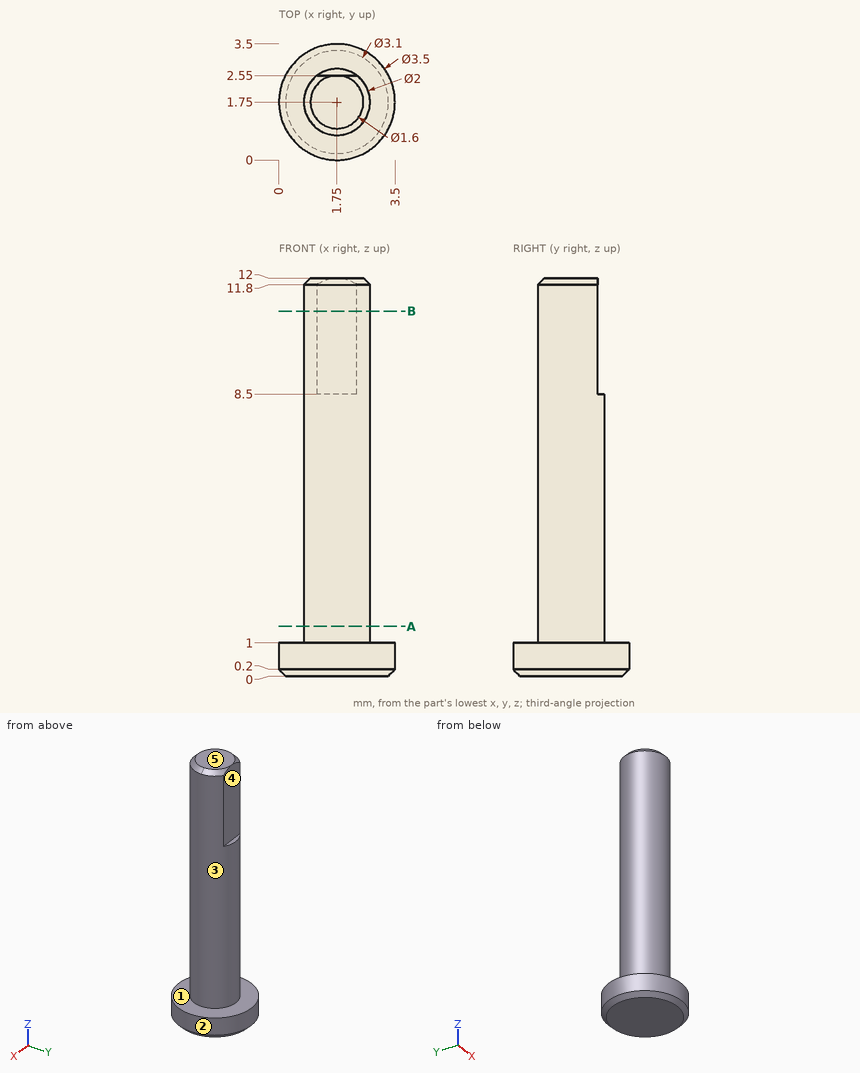
Design review of the part shown in the three views and the two pictorial views. Dimensions are in mm from the part's minimum x, y and z. A direction names the side the tool comes from. Round coordinates to 2 decimals unless told otherwise and drop trailing zeros. Loops run counter-clockwise (first coordinate to the right, second up) from the corner with the lowest first, then second, coordinate; pieces in that order, holes last. Notation, with made-up numbers: M 88,15.5 L 101,15.5 A35 ccw 101,53.5 Z; hole C -38.75,40 d10. An arc over 180 degrees is marked long. Answer as a JSON object with one key per item and string values.
Item 1: Wall thickness on L1, parallel to Y at x = 2.55, z = 8; L2, parallel to Z at x = 2.8, y = 1.35; L3, parallel to X at y = 1.65, z = 3.5: over which ranges is each line inside the solid? List them lowest first. Write a range as from..to.
Answer sheet:
{"L1": "y = 1.15..2.35", "L2": "z = 0..1", "L3": "x = 0.76..2.74"}
Item 2: Clearance check with flat-ended pins moving along their axes: P1, Ø1.5, axis at y = 1.5, z = 8, coming from the +X side; P2, Ø1, axis at x = 1.5, z = 10.5, coming from the +Y side. State where each tip first meets the part, or that it passes through.
Answer sheet:
{"P1": "stops at x = 2.75", "P2": "stops at y = 2.55"}
Item 3: Machinability: for the marked faces 1 and 2, which of the approach directions +Z, -Z, +X, -X, +Y, -Y give a long, thin tool a straight path to every point of the face, cutting with its end or side? Answer none if there is none.
Answer sheet:
{"face 1": "+Z", "face 2": "+Z, -Z"}
Item 4: We need section B-B on z = 11. Give the boundary of the cut face in (x, y), and give its area (3 significant figures).
Answer sheet:
{"outline": "M 1.15,2.55 A1 ccw long 2.35,2.55 Z", "area": "2.98 mm^2"}
Item 5: We need section A-A on z = 1.5. Give the boundary of the cut face in (x, y).
Answer sheet:
{"outline": "C 1.75,1.75 d2"}
Item 6: The part is to be moulded in two halves that separate along Y. For the marked faces 3, 4 and 5, say which applies: pulls with the +Y half, pulls with the -Y half, needs draft (parallel to the pull), parting line crosses it, or undercut.
Answer sheet:
{"face 3": "parting line crosses it", "face 4": "pulls with the +Y half", "face 5": "needs draft"}
